```python
from build123d import *

# Parameters (mm, degrees)
SKETCH_1_W             = 80
SKETCH_1_H             = 70
EXTRUDE_1_DEPTH        = 12.4
HOLE_WIZARD_M6_1_D     = 5
HOLE_WIZARD_M6_1_DEPTH = 15
HOLE_WIZARD_M6_1_TIP   = 1.502151548
HOLE_WIZARD_M6_2_D     = 5


with BuildPart() as part:
    # 草图1 → 凸台-拉伸1 (new body)
    with BuildSketch(Plane(origin=(0, 0, 0), x_dir=(0, 0, -1), z_dir=(1, 0, 0))):
        Rectangle(SKETCH_1_W, SKETCH_1_H)
    extrude(amount=EXTRUDE_1_DEPTH)

    # M6 螺纹孔1
    with Locations(Plane(origin=(12.4, 0, 0), x_dir=(0, 0, -1), z_dir=(1, 0, 0))):
        with Locations((-17.5, 28), (17.5, 28), (-17.5, -28), (17.5, -28)):
            Hole(HOLE_WIZARD_M6_1_D / 2, depth=HOLE_WIZARD_M6_1_DEPTH)
            with Locations((0, 0, -(HOLE_WIZARD_M6_1_DEPTH + HOLE_WIZARD_M6_1_TIP / 2))):  # 118° drill point
                Cone(0, HOLE_WIZARD_M6_1_D / 2, HOLE_WIZARD_M6_1_TIP, mode=Mode.SUBTRACT)

    # M6 螺纹孔2 (through all)
    with Locations(Plane(origin=(12.4, 0, 0), x_dir=(0, 0, -1), z_dir=(1, 0, 0))):
        with Locations((-33, 28), (-33, -28), (33, -28), (33, 28)):
            Hole(HOLE_WIZARD_M6_2_D / 2)


solid = part.part
```
Check sheet for the modelled part. Datum: model origin and axes. Units: mm. Coordinates: 2 decimals unless noted, no trailing zeros. Loops run counter-clockwise (first coordinate to the right, second up) from the corner with the lowest first, then second, coordinate; pieces in that order, holes last. Notation, with made-up numbers: M 84.25,7.25 L 112.25,7.25 A14 ccw 112.25,13.25 Z; hole C 0,78.5 d7. An arc over 180 degrees is marked long. Answer as a JSON object with one key per item and string values.
1. Release check for a two-part mould opening along Z. For faces 1 (the flat face through (6, 0, -40)), 2 (the flat face through (6, 35, 1)), 3 (the cylindrical face through (6.11, -25.52, 32.67)) record: pulls with the +Z half, pulls with the -Z half, needs draft (parallel to the pull), parting line crosses it, or undercut.
Outcome:
{"face 1": "pulls with the -Z half", "face 2": "needs draft", "face 3": "undercut"}
2. Depth check by flat-ended pin: P1, Ø3, axis at y = 28, z = -33, coming from the +X side; P2, Ø6, axis at y = -28, z = 17.5, coming from the -X side. Enter the tip coordinate at first touch or a pass-through.
Outcome:
{"P1": "through", "P2": "x = 0"}
3. Scan lines: L1, parallel to Y at x = 4, z = -17.5; L2, parallel to Z at x = 6, y = 26.5; L3, parallel to Y at x = 12, z = -18. Record each from-to range of solid material in increasing order. Write a range as from..to.
Outcome:
{"L1": "-35..-30.5, -25.5..25.5, 30.5..35", "L2": "-40..-35, -31..-19.5, -15.5..15.5, 19.5..31, 35..40", "L3": "-35..-30.45, -25.55..25.55, 30.45..35"}
4. Sectioned sample at C-C on y = 28. Record the cut outline in (x, z).
Outcome:
{"outline": "M 0,-40 L 12.4,-40 L 12.4,-35.5 L 0,-35.5 Z; M 0,-30.5 L 12.4,-30.5 L 12.4,-20 L 0,-20 Z; M 0,-15 L 12.4,-15 L 12.4,15 L 0,15 Z; M 0,20 L 12.4,20 L 12.4,30.5 L 0,30.5 Z; M 0,35.5 L 12.4,35.5 L 12.4,40 L 0,40 Z"}
5. Sectioned sample at D-D on z = -33. Record the cut outline in (x, y).
Outcome:
{"outline": "M 0,-35 L 12.4,-35 L 12.4,-30.5 L 0,-30.5 Z; M 0,-25.5 L 12.4,-25.5 L 12.4,25.5 L 0,25.5 Z; M 0,30.5 L 12.4,30.5 L 12.4,35 L 0,35 Z"}
6. Sectioned sample at A-A on x = 7.25. Count the separate pieces of the cut face and the enclosed holes in it, and give its area (3 significant figures).
Outcome:
{"separate pieces": "1", "enclosed holes": "8", "area": "5,440 mm²"}
7. Sectioned sample at B-B on z = 31.5. Record the cut outline in (x, y).
Outcome:
{"outline": "M 0,-35 L 12.4,-35 L 12.4,-30 L 0,-30 Z; M 0,-26 L 12.4,-26 L 12.4,26 L 0,26 Z; M 0,30 L 12.4,30 L 12.4,35 L 0,35 Z"}
